Check sheet for the drawn part. Datum: minimum x, y, z corner. Units: mm. A direction names the side the tool comes from. Coordinates: 2 decimals unless noted, no trailing zeros. Order: outer loops, then holes, each group sorted by start corner. A loop starts at its lowest first (then second) coordinate and runs counter-clockwise, first axis right, second up. Notation, with made-up numbers: (32.5, -37.75) -> (61.5, -37.75) arc R21 ccw to (61.5, -15.75) -> close; hole circle Ø5 at (2, 44.25). An arc over 180 degrees is marked (long way). Answer as CSV lines item,"result".
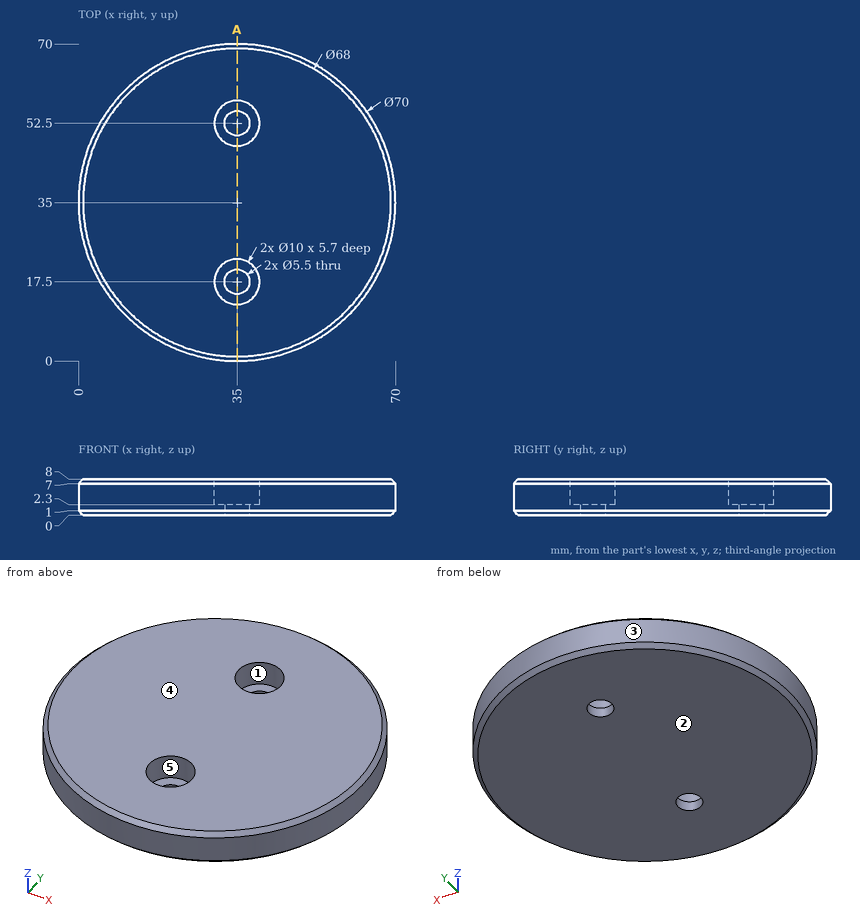
Item 1: Tool access check on the marked faces 1 and 2. Record the directions out of +Z, -Z, +X, -X, +Y, -Y that give a thin tool (end or side, any length) a straight path to the whole face; none if there is none.
Answer list:
face 1,"+Z"
face 2,"-Z, +X, -X, +Y, -Y"
Item 2: Thickness scan on line 1 (Y direction, x = 35, z = 3.6); line 2 (Y direction, x = 37, z = 5); line 3 (Z direction, x = 31.5, y = 17.5). Record the ranges inside material, lowest first.
Answer list:
line 1,"0 to 12.5, 22.5 to 47.5, 57.5 to 70"
line 2,"0.06 to 12.92, 22.08 to 47.92, 57.08 to 69.94"
line 3,"0 to 2.3"
Item 3: Depth check by flat-ended pin: pin 1 Ø8 at (x, y) = (35, 17.5) entering from +Z; pin 2 Ø8 at (x, y) = (35, 52.5) entering from -Z; pin 3 Ø2 at (y, z) = (61.5, 5) entering from +X; pin 4 Ø3 at (y, z) = (32.5, 5.5) entering from -X. Enter the tip coordinate at first touch or a pass-through.
Answer list:
pin 1,"z = 2.3"
pin 2,"z = 0"
pin 3,"x = 58.97"
pin 4,"x = 0.01"
Item 4: Release check for a two-part mould opening along Y. For the marked faces 3, 4 and 5 record: +Y half, -Y half, draft (parallel to the pull), parting line (faces both ways), or undercut.
Answer list:
face 3,"parting line"
face 4,"draft"
face 5,"undercut"
Item 5: Section check A-A, the plane x = 35. Record the boundary of the cut face in (y, z), plus the area to 3 significant figures.
Answer list:
outline,"(0, 1) -> (1, 0) -> (14.75, 0) -> (14.75, 2.3) -> (12.5, 2.3) -> (12.5, 8) -> (1, 8) -> (0, 7) -> close; (20.25, 0) -> (49.75, 0) -> (49.75, 2.3) -> (47.5, 2.3) -> (47.5, 8) -> (22.5, 8) -> (22.5, 2.3) -> (20.25, 2.3) -> close; (55.25, 0) -> (69, 0) -> (70, 1) -> (70, 7) -> (69, 8) -> (57.5, 8) -> (57.5, 2.3) -> (55.25, 2.3) -> close"
area,"419 mm2"
